Check sheet for the modelled part. Datum: model origin and axes. Units: mm. A direction names the side the tool comes from. Give positions to 0.01 mm unless a question says otherwise; leave off trailing zeros. Order: outer loops, then holes, each group sorted by start corner. A loop starts at its lowest first (then second) coordinate and runs counter-clockwise, first axis right, second up. Notation, with made-up numbers: (66.5, 5) - (92.5, 5) arc R30 ccw to (92.5, 28) - close; hole circle Ø6 at (-26.75, 6.5). An arc over 180 degrees is marked (long way). Answer in a Markdown table with one row per item.
from build123d import *

# Parameters (mm, degrees)
HUB_PROFILE_SKETCH_W        = 5
HUB_PROFILE_SKETCH_H        = 20
HUB_PROFILE_SKETCH_W_2      = 4
MOUNTING_HOLES_SKETCH_R     = 14
MOUNTING_HOLES_SKETCH_R_2   = 2.65
MOUNTING_HOLES_4X_5_3_DEPTH = 317
SLOT_SKETCH_R               = 3.5
SLOT_7MM_X_4_DEEP_DEPTH     = 4
RECESS_SKETCH_R             = 19
RECESS_38_X_6_DEEP_DEPTH    = 6


with BuildPart() as part:
    # Hub Profile Sketch → Flanged Hub Body (revolve)
    with BuildSketch(Plane.XY, mode=Mode.PRIVATE) as flanged_hub_body_sk:
        with BuildLine():
            Line((-5, -19), (0, -19))
            Line((0, -19), (4.6, -19))
            ThreePointArc((4.6, -19), (6.014213562, -18.414213562), (6.6, -17))
            Line((6.6, -17), (6.6, 0))
            Line((6.6, 0), (-9, 0))
            Line((-9, 0), (-9, -19))
            Line((-9, -19), (-5, -19))
        make_face()
        with BuildLine():
            Line((9, -39), (9, -24))
            Line((9, -24), (21.4, -24))
            Line((21.4, -24), (21.4, 0))
            Line((21.4, 0), (6.6, 0))
            Line((6.6, 0), (6.6, -17))
            ThreePointArc((6.6, -17), (6.014213562, -18.414213562), (4.6, -19))
            Line((4.6, -19), (0, -19))
            Line((0, -19), (0, -39))
            Line((0, -39), (9, -39))
        make_face()
        with Locations((-2.5, -29)):
            Rectangle(HUB_PROFILE_SKETCH_W, HUB_PROFILE_SKETCH_H)
        with Locations((-7, -29)):
            Rectangle(HUB_PROFILE_SKETCH_W_2, HUB_PROFILE_SKETCH_H)
    revolve(flanged_hub_body_sk.sketch.rotate(Axis((6.6, 0, 0), (1, 0, 0)), 270), axis=Axis((6.6, 0, 0), (1, 0, 0)))

    # Mounting Holes Sketch → Mounting Holes 4xØ5.3 (cut)
    with BuildSketch(Plane(origin=(21.4, 0, 0), x_dir=(0, 0, -1), z_dir=(1, 0, 0))):
        Circle(MOUNTING_HOLES_SKETCH_R)
        with Locations(Location((0, 32.26943336, 0), (0, 0, 180))):
            Circle(MOUNTING_HOLES_SKETCH_R_2)
        with Locations(Location((32.26943336, 0, 0), (0, 0, 180))):
            Circle(MOUNTING_HOLES_SKETCH_R_2)
        with Locations(Location((0, -32.26943336, 0), (0, 0, 180))):
            Circle(MOUNTING_HOLES_SKETCH_R_2)
        with Locations(Location((-32.26943336, 0, 0), (0, 0, 180))):
            Circle(MOUNTING_HOLES_SKETCH_R_2)
    extrude(amount=-MOUNTING_HOLES_4X_5_3_DEPTH, mode=Mode.SUBTRACT)

    # Slot Sketch → Slot 7mm x 4 Deep (cut)
    with BuildSketch(Plane.ZY.offset(9)):
        with Locations((0, 32.26943336)):
            Circle(SLOT_SKETCH_R)
        with Locations((-32.26943336, 0)):
            Circle(SLOT_SKETCH_R)
        with Locations((0, -32.26943336)):
            Circle(SLOT_SKETCH_R)
        with Locations((32.26943336, 0)):
            Circle(SLOT_SKETCH_R)
    extrude(amount=-SLOT_7MM_X_4_DEEP_DEPTH, mode=Mode.SUBTRACT)

    # Recess Sketch → Recess Ø38 x 6 Deep (cut)
    with BuildSketch(Plane.ZY.offset(9)):
        Circle(RECESS_SKETCH_R)
    extrude(amount=-RECESS_38_X_6_DEEP_DEPTH, mode=Mode.SUBTRACT)


solid = part.part
(1) Access from +Z, -Z, +X, -X, +Y, -Y to the whole of each face (thin tool, end or side, straight path). Record for faces 4 (the cylindrical face through (2.098, -0.796, -29.742)), 5 (the cylindrical face through (-7.03, 1.05, -28.93)).
Geometry says:
| item | result |
|---|---|
| face 4 | +X, -X |
| face 5 | -X |
(2) Cross-section at C-C, the plane x = 17.5. Record the cut outline in (y, z), then the cut area to 3 significant figures.
Geometry says:
| item | result |
|---|---|
| outline | circle Ø48 at (0, 0); hole circle Ø28 at (0, 0) |
| area | 1,190 mm² |
(3) Mould release check, pull along Y, two halves, no side actions. Record for faces 1 (the flat face through (-5, -31, -3)), 2 (the flat face through (21.4, 10.3, 10.3)), 3 (the cylindrical face through (15.29, -7.21, 22.89)): pulls with the +Y half, pulls with the -Y half, needs draft (parallel to the pull), parting line crosses it, or undercut.
Geometry says:
| item | result |
|---|---|
| face 1 | undercut |
| face 2 | needs draft |
| face 3 | parting line crosses it |
(4) Thickness scan on L1, parallel to Y at x = 7, z = 0; L2, parallel to Y at x = 11.5, z = 0; L3, parallel to Y at x = -4, z = 7. Record the ranges inside material, lowest first.
Geometry says:
| item | result |
|---|---|
| L1 | -39 to -34.92, -29.62 to -14, 14 to 29.62, 34.92 to 39 |
| L2 | -24 to -14, 14 to 24 |
| L3 | -38.37 to -17.66, 17.66 to 38.37 |
(5) Gauge pin test, flat ends, axial feed: P1, Ø11.5, axis at y = -9, z = 6, coming from the -X side; P2, Ø7, axis at y = 0, z = -32.27, coming from the +X side; P3, Ø8, axis at x = 8.5, y = -17, coming from the +Z side. Record the tip position at first contact, or that the pin passes through.
Geometry says:
| item | result |
|---|---|
| P1 | x = -3 |
| P2 | x = 9 |
| P3 | z = 36.77 |
(6) Cross-section at D-D, the plane z = -17.5. Record the cut outline in (x, y).
Geometry says:
| item | result |
|---|---|
| outline | (-9, -34.85) - (9, -34.85) - (9, -16.42) - (21.4, -16.42) - (21.4, 16.42) - (9, 16.42) - (9, 34.85) - (-9, 34.85) - (-9, 7.4) - (-3, 7.4) - (-3, -7.4) - (-9, -7.4) - close |
(7) Cross-section at A-A, the plane y = 0. Give the number of separate pieces and of enclosed holes in the cut face, then the cut area to 3 significant figures.
Geometry says:
| item | result |
|---|---|
| separate pieces | 4 |
| enclosed holes | 0 |
| area | 884 mm² |
